The model under review builds one solid part; all positions refer to its coordinate system, in mm. Face numbers are marked on the shaded views. A direction names the side the tool comes from. Round coordinates to 2 decimals unless told otherwise and drop trailing zeros. Loops run counter-clockwise (first coordinate to the right, second up) from the corner with the lowest first, then second, coordinate; pieces in that order, holes last. Notation, with made-up numbers: M 65.25,81.25 L 110.25,81.25 A30 cw 110.25,112.25 Z; hole C 41,43 d11. An arc over 180 degrees is marked long. Answer as a JSON object with one key per item and string values. Group by question number.
Item 1: Consider section A-A (z = 2.35). State how many separate pieces and enclosed holes the cut face has, and give its area (3 significant figures).
Item 2: Insertion check: P1, Ø2.5, axis at x = 11.1, y = 12, coming from the +Z side; P2, Ø7, axis at x = 15, y = 10, coming from the +Z side; P3, Ø2.5, axis at x = 18, z = 1, coming from the +Y side; P4, Ø4.5, axis at x = 17, y = 7, coming from the +Z side. Each pin has a flat end and moves straight along its axis. Give the tip position at first contact, or say it passes through.
Item 3: Tool access review of the marked faces 1, 2 and 3: name each direction out of +Z, -Z, +X, -X, +Y, -Y from which nothing blocks a thin tool from reaching the whole face with its end or side.
Item 4: To check wall thickness, follow line 1 (Y direction, x = 3, z = 2.95); line 2 (Y direction, x = 9.5, z = 2.4); line 3 (Y direction, x = 35.5, z = 2.4). State the ranges of each line that lie inside material, in increasing order.
Item 5: The part is to be moulded in two halves that separate along X. For the marked faces 4, 5, 6 and 7, say which applies: +X half, -X half, draft (parallel to the pull), parting line (faces both ways), or undercut.
Item 6: Consider section B-B (x = 6.5). Give the boundary of the cut face in (y, z), and give its area (3 significant figures).
Item 7: Consider section D-D (z = 3.95). Give the boundary of the cut face in (x, y).
Item 8: Consider section C-C (y = 4.5). Give the boundary of the cut face in (x, z).
```python
from build123d import *

# Parameters (mm, degrees)
BASE_PLATE_DEPTH         = 2
PERIMETER_RIM_DEPTH      = 1
PIN_1_SKETCH_R           = 1
PIN_1_2_DEPTH            = 4
PIN_2_SKETCH_R           = 1
PIN_2_2_DEPTH            = 4
THROUGH_HOLES_SKETCH_R   = 1.5
THROUGH_HOLES_3X_3_DEPTH = 4


with BuildPart() as part:
    # Base Plate Sketch → Base Plate (new body)
    with BuildSketch(Plane.XY):
        with BuildLine():
            Line((0, 3), (0, 12))
            ThreePointArc((0, 12), (0.878679656, 14.121320344), (3, 15))
            Line((3, 15), (11.101020514, 15))
            ThreePointArc((11.101020514, 15), (12.998387111, 14.323790008), (14.040408206, 12.6))
            ThreePointArc((14.040408206, 12.6), (14.735088936, 11.450806662), (16, 11))
            Line((16, 11), (22, 11))
            ThreePointArc((22, 11), (23.414213562, 11.585786438), (24, 13))
            Line((24, 13), (32, 13))
            ThreePointArc((32, 13), (32.585786438, 11.585786438), (34, 11))
            Line((34, 11), (36, 11))
            ThreePointArc((36, 11), (38.121320344, 10.121320344), (39, 8))
            Line((39, 8), (39, 3))
            ThreePointArc((39, 3), (38.121320344, 0.878679656), (36, 0))
            Line((36, 0), (3, 0))
            ThreePointArc((3, 0), (0.878679656, 0.878679656), (0, 3))
        make_face()
    extrude(amount=BASE_PLATE_DEPTH)

    # Perimeter Rim Sketch → Perimeter Rim (add)
    with BuildSketch(Plane.XY.offset(2)):
        with BuildLine():
            Line((32, 13), (24, 13))
            ThreePointArc((24, 13), (23.414213562, 11.585786438), (22, 11))
            Line((22, 11), (16, 11))
            ThreePointArc((16, 11), (14.735088936, 11.450806662), (14.040408206, 12.6))
            ThreePointArc((14.040408206, 12.6), (12.998387111, 14.323790008), (11.101020514, 15))
            Line((11.101020514, 15), (3, 15))
            ThreePointArc((3, 15), (0.878679656, 14.121320344), (0, 12))
            Line((0, 12), (0, 3))
            ThreePointArc((0, 3), (0.878679656, 0.878679656), (3, 0))
            Line((3, 0), (36, 0))
            ThreePointArc((36, 0), (38.121320344, 0.878679656), (39, 3))
            Line((39, 3), (39, 8))
            ThreePointArc((39, 8), (38.121320344, 10.121320344), (36, 11))
            Line((36, 11), (34, 11))
            ThreePointArc((34, 11), (32.585786438, 11.585786438), (32, 13))
        make_face()
        with BuildLine():
            Line((31.763932023, 12.75), (24.236067977, 12.75))
            ThreePointArc((24.236067977, 12.75), (23.5, 11.322949017), (22, 10.75))
            Line((22, 10.75), (16, 10.75))
            ThreePointArc((16, 10.75), (14.576975053, 11.257157494), (13.795459231, 12.55))
            ThreePointArc((13.795459231, 12.55), (12.840273228, 14.13014084), (11.101020514, 14.75))
            Line((11.101020514, 14.75), (3, 14.75))
            ThreePointArc((3, 14.75), (1.055456352, 13.944543648), (0.25, 12))
            Line((0.25, 12), (0.25, 3))
            ThreePointArc((0.25, 3), (1.055456352, 1.055456352), (3, 0.25))
            Line((3, 0.25), (36, 0.25))
            ThreePointArc((36, 0.25), (37.944543648, 1.055456352), (38.75, 3))
            Line((38.75, 3), (38.75, 8))
            ThreePointArc((38.75, 8), (37.944543648, 9.944543648), (36, 10.75))
            Line((36, 10.75), (34, 10.75))
            ThreePointArc((34, 10.75), (32.5, 11.322949017), (31.763932023, 12.75))
        make_face(mode=Mode.SUBTRACT)
    extrude(amount=PERIMETER_RIM_DEPTH)

    # Pin 1 Sketch → Pin 1 Ø2 (add)
    with BuildSketch(Plane.XY.offset(2)):
        with Locations((36, 3)):
            Circle(PIN_1_SKETCH_R)
    extrude(amount=PIN_1_2_DEPTH)

    # Pin 2 Sketch → Pin 2 Ø2 (add)
    with BuildSketch(Plane.XY.offset(2)):
        with Locations((3, 12)):
            Circle(PIN_2_SKETCH_R)
    extrude(amount=PIN_2_2_DEPTH)

    # Through Holes Sketch → Through Holes 3xØ3 (cut)
    with BuildSketch(Plane.XY.offset(2)):
        with Locations((36, 8)):
            Circle(THROUGH_HOLES_SKETCH_R)
        with Locations((11.101020514, 12)):
            Circle(THROUGH_HOLES_SKETCH_R)
        with Locations((7.101020514, 12)):
            Circle(THROUGH_HOLES_SKETCH_R)
    extrude(amount=-THROUGH_HOLES_3X_3_DEPTH, mode=Mode.SUBTRACT)


solid = part.part
```
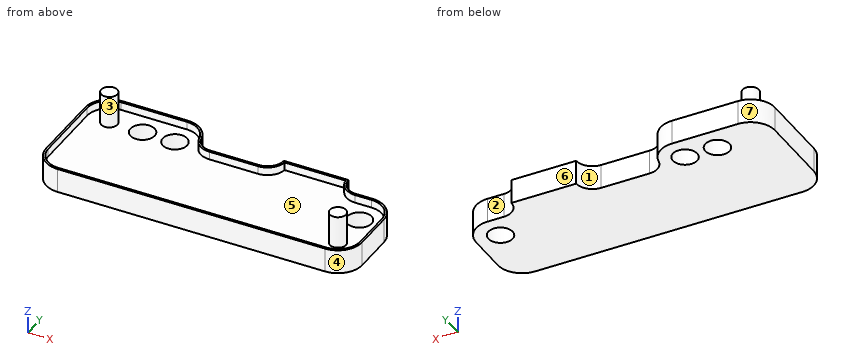
Geometry results:
{
 "1": {"separate pieces": "3", "enclosed holes": "1", "area": "31.8 mm^2"},
 "2": {"P1": "passes through", "P2": "stops at z = 3", "P3": "stops at y = 11", "P4": "stops at z = 2"},
 "3": {"face 1": "+Z, -Z, +Y", "face 2": "+Z, -Z, +X, +Y", "face 3": "+Z"},
 "4": {"line 1": "y = 0 to 0.25, 11 to 13, 14.75 to 15", "line 2": "y = 0 to 0.25, 14.75 to 15", "line 3": "y = 0 to 0.25, 2.13 to 3.87, 10.75 to 11"},
 "5": {"face 4": "+X half", "face 5": "undercut", "face 6": "draft", "face 7": "-X half"},
 "6": {"outline": "M 0,0 L 10.63,0 L 10.63,2 L 0.25,2 L 0.25,3 L 0,3 Z; M 13.37,0 L 15,0 L 15,3 L 14.75,3 L 14.75,2 L 13.37,2 Z", "area": "25.0 mm^2"},
 "7": {"outline": "C 3,12 d2; C 36,3 d2"},
 "8": {"outline": "M 0,0 L 39,0 L 39,3 L 38.75,3 L 38.75,2 L 0.25,2 L 0.25,3 L 0,3 Z"}
}
